Could you check a few things on this model? Use its own coordinates, in mm. A direction names the side the tool comes from. Give positions to 0.01 mm unless a question says otherwise; leave off trailing zeros. Loops run counter-clockwise (first coordinate to the right, second up) from the corner with the lowest first, then second, coordinate; pieces in that order, holes last. Notation, with made-up numbers: (33.25, 52.25) - (37.25, 52.25) arc R31 cw to (37.25, 84.25) - close; hole circle Ø3 at (25.25, 67). An arc over 180 degrees is marked (long way). Write each question's results on one line, items separated by ' | '. Start each with the question number.
```python
from build123d import *

# Parameters (mm, degrees)
EXTRUDE_1_DEPTH = 15


with BuildPart() as part:
    # 草图1 → 凸台-拉伸1 (new, symmetric)
    with BuildSketch(Plane.XY):
        Polygon((0, 0), (70, 0), (70, 6), (6, 6), (6, 74), (0, 74), align=None)
    extrude(amount=EXTRUDE_1_DEPTH, both=True)


solid = part.part
```
Q1. I want a section at A-A, the plane z = -5. List the corners of the cut face in (x, y) for me, then the cut area to 3 significant figures.
Q2. I'm going to push flat-ended pins straight in: pin 1 Ø8 at (y, z) = (25, 6) entering from -X; pin 2 Ø10 at (x, y) = (22.5, 12.5) entering from -Z; pin 3 Ø5 at (x, z) = (42.5, -4) entering from +Y; pin 4 Ø10 at (y, z) = (58.5, -3) entering from +X. Where does each tip first touch, or does it pass through?
Q3. I want a section at B-B, the plane y = 9.5. List the corners of the cut face in (x, z) for me.
Q4. Which directions (+Z, -Z, +X, -X, +Y, -Y) give clear straight access to the entire face, cutting with the end or side of a thin tool? Please do faces 1 (the face through (70, 3, 0)), 2 (the face through (38, 6, 0)).
Q5. I need wall thicknesses on L1, parallel to X at y = 19, z = -12. Which ranges of the line are inside material? Lowest first, please. Write a range as from..to.
Conclusion:
1) outline: (0, 0) - (70, 0) - (70, 6) - (6, 6) - (6, 74) - (0, 74) - close | area: 828 mm^2
2) pin 1: x = 0 | pin 2: through | pin 3: y = 6 | pin 4: x = 6
3) outline: (0, -15) - (6, -15) - (6, 15) - (0, 15) - close
4) face 1: +Z, -Z, +X, +Y, -Y | face 2: +Z, -Z, +X, +Y
5) L1: 0..6
